For this review, take the finished solid that the model builds, in its own axes (mm). Give positions to 0.01 mm unless a question says otherwise; leave off trailing zeros. Write each loop counter-clockwise with the first axis right and the second up, starting at its lowest first coordinate (ties: lowest second). Pieces come first, ordered by that corner, then holes. Notation, with made-up numbers: (-9.75, 32) -> (35.25, 32) arc R37 ccw to (35.25, 68) -> close; hole circle Ø1 at (31, 66). An arc over 180 degrees is marked (long way). Return JSON: item names as keys, results as strings.
from build123d import *

# Parameters (mm, degrees)
SKETCH_1_R      = 7.5
SKETCH_1_R_2    = 1.55
EXTRUDE_1_DEPTH = 2
FILLET_1_R      = 2


with BuildPart() as part:
    # 草图1 → 凸台-拉伸1 (new body)
    with BuildSketch(Plane(origin=(0, 0, 0), x_dir=(1, 0, 0), z_dir=(0, 1, 0))):
        with BuildLine():
            Line((17.081451175, -20.909902577), (-17.081451175, -20.909902577))
            ThreePointArc((-17.081451175, -20.909902577), (-19.091883092, -19.091883092), (-20.909902577, -17.081451175))
            Line((-20.909902577, -17.081451175), (-20.909902577, 17.081451175))
            ThreePointArc((-20.909902577, 17.081451175), (-19.091883092, 19.091883092), (-17.081451175, 20.909902577))
            Line((-17.081451175, 20.909902577), (17.081451175, 20.909902577))
            ThreePointArc((17.081451175, 20.909902577), (19.091883092, 19.091883092), (20.909902577, 17.081451175))
            Line((20.909902577, 17.081451175), (20.909902577, -17.081451175))
            ThreePointArc((20.909902577, -17.081451175), (19.091883092, -19.091883092), (17.081451175, -20.909902577))
        make_face()
        with Locations(Location((0, 0, 0), (0, 0, 270))):
            Circle(SKETCH_1_R, mode=Mode.SUBTRACT)
        with Locations(Location((12, 0, 0), (0, 0, 270))):
            Circle(SKETCH_1_R_2, mode=Mode.SUBTRACT)
        with Locations(Location((15.909902577, 15.909902577, 0), (0, 0, 270))):
            Circle(SKETCH_1_R_2, mode=Mode.SUBTRACT)
        with Locations(Location((0, -12, 0), (0, 0, 270))):
            Circle(SKETCH_1_R_2, mode=Mode.SUBTRACT)
        with Locations(Location((15.909902577, -15.909902577, 0), (0, 0, 270))):
            Circle(SKETCH_1_R_2, mode=Mode.SUBTRACT)
        with Locations(Location((-12, 0, 0), (0, 0, 270))):
            Circle(SKETCH_1_R_2, mode=Mode.SUBTRACT)
        with Locations(Location((-15.909902577, -15.909902577, 0), (0, 0, 270))):
            Circle(SKETCH_1_R_2, mode=Mode.SUBTRACT)
        with Locations(Location((0, 12, 0), (0, 0, 270))):
            Circle(SKETCH_1_R_2, mode=Mode.SUBTRACT)
        with Locations(Location((-15.909902577, 15.909902577, 0), (0, 0, 270))):
            Circle(SKETCH_1_R_2, mode=Mode.SUBTRACT)
    extrude(amount=EXTRUDE_1_DEPTH)

    # 圆角1
    fillet_1_edges = [part.edges().sort_by_distance(p)[0] for p in [
        (17.081451175, 1, 20.909902577),
        (-17.081451175, 1, 20.909902577),
        (-20.909902577, 1, 17.081451175),
        (-20.909902577, 1, -17.081451175),
        (-17.081451175, 1, -20.909902577),
        (17.081451175, 1, -20.909902577),
        (20.909902577, 1, -17.081451175),
        (20.909902577, 1, 17.081451175),
    ]]
    fillet(fillet_1_edges, radius=FILLET_1_R)


solid = part.part
1. Add section B-B, the plane x = 0. State the section outline as (y, z) points.
Results found:
{"outline": "(0, -20.91) -> (2, -20.91) -> (2, -13.55) -> (0, -13.55) -> close; (0, -10.45) -> (2, -10.45) -> (2, -7.5) -> (0, -7.5) -> close; (0, 7.5) -> (2, 7.5) -> (2, 10.45) -> (0, 10.45) -> close; (0, 13.55) -> (2, 13.55) -> (2, 20.91) -> (0, 20.91) -> close"}
2. Add section D-D, the plane z = -12. State the section outline as (x, y) points.
Results found:
{"outline": "(-20.91, 0) -> (-1.55, 0) -> (-1.55, 2) -> (-20.91, 2) -> close; (1.55, 0) -> (20.91, 0) -> (20.91, 2) -> (1.55, 2) -> close"}
3. Add section A-A, the plane z = 0. State the section outline as (x, y) points.
Results found:
{"outline": "(-20.91, 0) -> (-13.55, 0) -> (-13.55, 2) -> (-20.91, 2) -> close; (-10.45, 0) -> (-7.5, 0) -> (-7.5, 2) -> (-10.45, 2) -> close; (7.5, 0) -> (10.45, 0) -> (10.45, 2) -> (7.5, 2) -> close; (13.55, 0) -> (20.91, 0) -> (20.91, 2) -> (13.55, 2) -> close"}
4. The part is to be moulded in two halves that separate along Z. For faces 1 (the cylindrical face through (17.06, 1.01, -20.78)), 2 (the cylindrical face through (-16.504, 0.986, -14.478)), 3 (the cylindrical face through (20.78, 1.01, 17.06)), say which applies: +Z half, -Z half, draft (parallel to the pull), parting line (faces both ways), or undercut.
Results found:
{"face 1": "-Z half", "face 2": "undercut", "face 3": "+Z half"}
5. To check wall thickness, follow probe 1 along Z at (x, y) = (-16, 1.6); probe 2 along X at (y, z) = (0.4, 0); probe 3 along X at (y, z) = (0.8, 15). State the ranges of each line that lie inside material, in increasing order.
Results found:
{"probe 1": "z = -20.91 to -17.46, -14.36 to 14.36, 17.46 to 20.91", "probe 2": "x = -20.91 to -13.55, -10.45 to -7.5, 7.5 to 10.45, 13.55 to 20.91", "probe 3": "x = -20.91 to -17.16, -14.66 to 14.66, 17.16 to 20.91"}
6. Add section C-C, the plane x = -12. State the section outline as (y, z) points, plus the area to 3 significant figures.
Results found:
{"outline": "(0, -20.91) -> (2, -20.91) -> (2, -1.55) -> (0, -1.55) -> close; (0, 1.55) -> (2, 1.55) -> (2, 20.91) -> (0, 20.91) -> close", "area": "77.4 mm²"}
